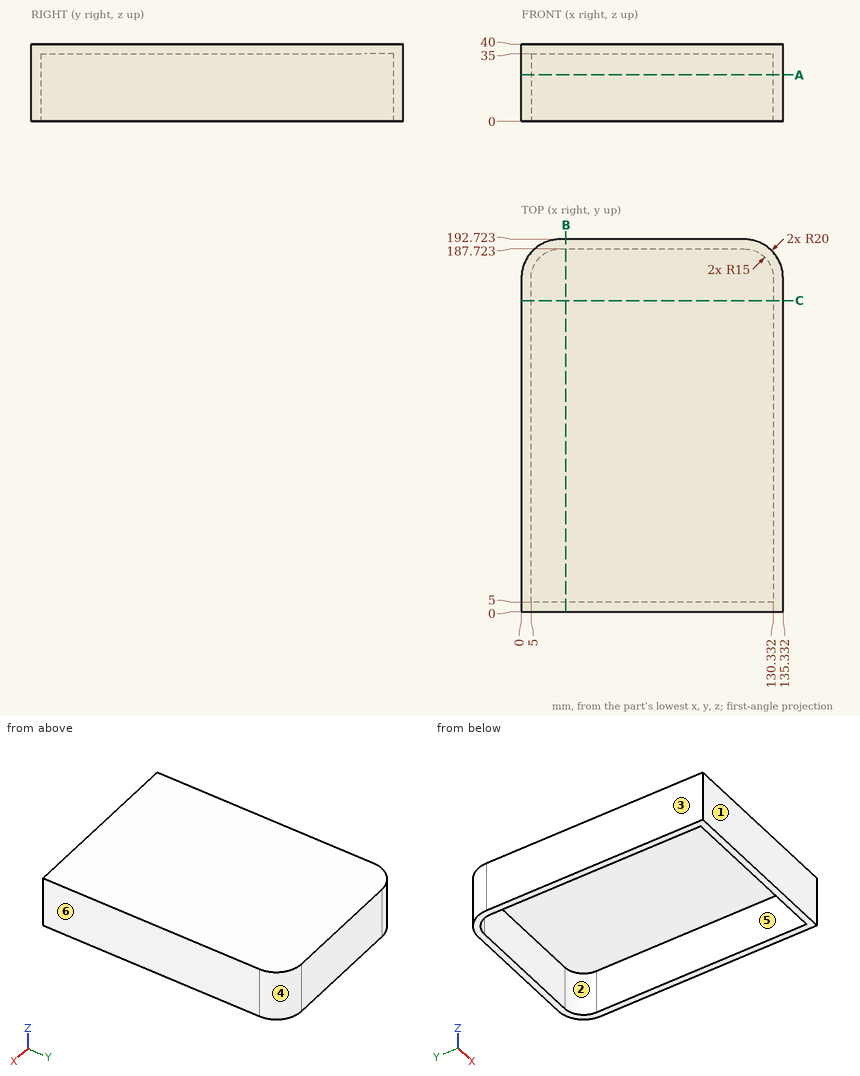
Could you check a few things on this drawing? It's one solid part, dimensions in mm from its lowest x, y, z. A direction names the side the tool comes from. Give positions to 0.01 mm unless a question says otherwise; leave off trailing zeros. Write each loop counter-clockwise with the first axis right and the second up, starting at its lowest first coordinate (ties: lowest second). Pieces come first, ordered by that corner, then holes. Notation, with made-up numbers: (58.25, -37) -> (73.25, -37) arc R28 ccw to (73.25, -18) -> close; hole circle Ø11 at (-0.75, 2.25). An arc over 180 degrees is marked (long way). Answer as CSV lines item,"result". Start each with the question number.
(1) Which directions (+Z, -Z, +X, -X, +Y, -Y) give clear straight access to the entire face, cutting with the end or side of a thin tool? Please do the marked faces 5 and 6.
(2) If we section it at C-C, the plane y = 161: Write out the boundary of the cut face in (x, z).
(3) If we section it at A-A, the plane z = 24: Write out the boundary of the cut face in (x, y).
(4) If we mould it in two halves opening along Y, with no side actions, what happens to the marked faces 1, 2, 3 and 4? For each: +Y half, -Y half, draft (parallel to the pull), parting line (faces both ways), or undercut.
(5) I'm going to push a flat-ended pin straight in: pin 1 Ø3 at (x, y) = (91, 87.5) entering from -Z. Where does the tip first touch, or does it pass through?
(6) If we section it at B-B, the plane x = 23: Write out the boundary of the cut face in (y, z), and give its area (3 significant figures).
(7) Please list where these lines run through material, in increasing order: line 1 (Y direction, x = 86, z = 33.5); line 2 (X direction, y = 64, z = 20.5); line 3 (Z direction, x = 104.5, y = 29).
Answer list:
1,face 5,"-Z"
1,face 6,"+Z, -Z, +X, +Y, -Y"
2,outline,"(0, 0) -> (5, 0) -> (5, 35) -> (130.33, 35) -> (130.33, 0) -> (135.33, 0) -> (135.33, 40) -> (0, 40) -> close"
3,outline,"(0, 0) -> (135.33, 0) -> (135.33, 172.72) arc R20 ccw to (115.33, 192.72) -> (20, 192.72) arc R20 ccw to (0, 172.72) -> close; hole (5, 5) -> (130.33, 5) -> (130.33, 172.72) arc R15 ccw to (115.33, 187.72) -> (20, 187.72) arc R15 ccw to (5, 172.72) -> close"
4,face 1,"-Y half"
4,face 2,"undercut"
4,face 3,"draft"
4,face 4,"+Y half"
5,pin 1,"z = 35"
6,outline,"(0, 0) -> (5, 0) -> (5, 35) -> (187.72, 35) -> (187.72, 0) -> (192.72, 0) -> (192.72, 40) -> (0, 40) -> close"
6,area,"1,310 mm^2"
7,line 1,"0 to 5, 187.72 to 192.72"
7,line 2,"0 to 5, 130.33 to 135.33"
7,line 3,"35 to 40"
